```python
from build123d import *

# Parameters (mm, degrees)
SKETCH2_R           = 14.5
BOSS_EXTRUDE1_DEPTH = 14
SKETCH3_W           = 4
SKETCH3_H           = 27
BOSS_EXTRUDE2_DEPTH = 12.3
CUT_EXTRUDE1_DEPTH  = 12.3
SKETCH5_R           = 11
BOSS_EXTRUDE3_DEPTH = 4
SKETCH6_W           = 29
SKETCH6_H           = 36.6
BOSS_EXTRUDE4_DEPTH = 50
FILLET1_R           = 0.2


with BuildPart() as part:
    # Sketch2 → Boss-Extrude1 (new body)
    with BuildSketch(Plane(origin=(0, 0, 0), x_dir=(1, 0, 0), z_dir=(0, 1, 0))):
        with Locations(Location((0, 0, 0), (0, 0, 270))):
            Circle(SKETCH2_R)
    extrude(amount=BOSS_EXTRUDE1_DEPTH)

    # Sketch3 → Boss-Extrude2 (add)
    with BuildSketch(Plane(origin=(0, 14, 0), x_dir=(1, 0, 0), z_dir=(0, 1, 0))):
        Rectangle(SKETCH3_W, SKETCH3_H)
    extrude(amount=BOSS_EXTRUDE2_DEPTH)

    # Sketch4 → Cut-Extrude1 (cut)
    with BuildSketch(Plane(origin=(2, 0, 0), x_dir=(0, 0, -1), z_dir=(1, 0, 0))):
        Polygon((-13.5, 26.3), (-13.5, 14), (-11, 26.3), align=None)
        Polygon((11, 26.3), (13.5, 26.3), (13.5, 14), align=None)
    extrude(amount=-CUT_EXTRUDE1_DEPTH, mode=Mode.SUBTRACT)

    # Sketch5 → Boss-Extrude3 (add)
    with BuildSketch(Plane.XZ):
        with Locations(Location((0, 0, 0), (0, 0, 90))):
            Circle(SKETCH5_R)
    extrude(amount=BOSS_EXTRUDE3_DEPTH)

    # Sketch6 → Boss-Extrude4 (add)
    with BuildSketch(Plane.XZ.offset(4)):
        Rectangle(SKETCH6_W, SKETCH6_H)
    extrude(amount=BOSS_EXTRUDE4_DEPTH)

    # Fillet1
    fillet1_edges = [part.edges().sort_by_distance(p)[0] for p in [
        (2, 26.3, 0),
        (-2, 20.15, 12.25),
        (2, 20.15, 12.25),
        (-2, 26.3, 0),
        (-2, 20.15, -12.25),
        (2, 20.15, -12.25),
        (0, 14, -14.5),
    ]]
    fillet(fillet1_edges, radius=FILLET1_R)


solid = part.part
```
Verification items for the finished model (mm, model axes). A direction names the side the tool comes from. Coordinates: 2 decimals unless noted, no trailing zeros. Order: outer loops, then holes, each group sorted by start corner. A loop starts at its lowest first (then second) coordinate and runs counter-clockwise, first axis right, second up. Notation, with made-up numbers: (-37, -23.75) - (-18, -23.75) arc R22 ccw to (-18, -4.75) - close; hole circle Ø11 at (61, -4.75). An arc over 180 degrees is marked (long way). Return JSON: item names as keys, results as strings.
(1) Go/stop test with flat-tipped pins: pin 1 (3 mm diameter, centred on y = -0.5, z = 10.5, fed in from -X); pin 2 (9.5 mm diameter, centred on y = 19.5, z = 1.5, fed in from -X); pin 3 (9.5 mm diameter, centred on y = 19.5, z = 5.5, fed in from +X). Record where each tip stops, or that it passes through.
Filled sheet:
{"pin 1": "stops at x = -11.3", "pin 2": "stops at x = -2", "pin 3": "stops at x = 2"}
(2) Section check A-A, the plane x = 0. Record the cut outline in (y, z), and give its area (3 significant figures).
Filled sheet:
{"outline": "(-54, -18.3) - (-4, -18.3) - (-4, -11) - (0, -11) - (0, -14.5) - (13.8, -14.5) arc R0.2 ccw to (14, -14.3) - (14, -13.5) - (26.3, -11) - (26.3, 11) - (14, 13.5) - (14, 14.3) arc R0.2 ccw to (13.8, 14.5) - (0, 14.5) - (0, 11) - (-4, 11) - (-4, 18.3) - (-54, 18.3) - close", "area": "2,630 mm^2"}
(3) Access from +Z, -Z, +X, -X, +Y, -Y to the whole of each face (thin tool, end or side, straight path). Record for faces 1 (the flat face through (11, 0, -2)), 2 (the flat face through (0.03, 20.06, 12.27)), 3 (the cylindrical face through (-5.554, 6.803, 13.394)), 4 (the flat face through (0.03, 20.06, -12.27)), 5 (the flat face through (2, 20, 0)).
Filled sheet:
{"face 1": "none", "face 2": "+Z, +X, -X, +Y", "face 3": "+Y", "face 4": "-Z, +X, -X, +Y", "face 5": "+Z, -Z, +X, +Y"}
(4) Section check B-B, the plane z = 0. Record the cut outline in (x, y), and give its area (3 significant figures).
Filled sheet:
{"outline": "(-14.5, -54) - (14.5, -54) - (14.5, -4) - (11, -4) - (11, 0) - (14.5, 0) - (14.5, 13.8) arc R0.2 ccw to (14.3, 14) - (2, 14) - (2, 26.1) arc R0.2 ccw to (1.8, 26.3) - (-1.8, 26.3) arc R0.2 ccw to (-2, 26.1) - (-2, 14) - (-14.3, 14) arc R0.2 ccw to (-14.5, 13.8) - (-14.5, 0) - (-11, 0) - (-11, -4) - (-14.5, -4) - close", "area": "1,990 mm^2"}
(5) Mould release check, pull along Y, two halves, no side actions. Record for faces 6 (the flat face through (0, -4, -12)), 7 (the flat face through (-3, 14, 0)), 8 (the flat face through (-2, 20, 0)): pulls with the +Y half, pulls with the -Y half, needs draft (parallel to the pull), parting line crosses it, or undercut.
Filled sheet:
{"face 6": "undercut", "face 7": "pulls with the +Y half", "face 8": "needs draft"}
(6) Thickness scan on line 1 along Y through (x, z) = (-8.5, 7.5); line 2 along Y through (x, z) = (-6.5, 15); line 3 along Y through (x, z) = (4, 10). Record the ranges inside material, lowest first.
Filled sheet:
{"line 1": "y = -54 to -4, 0 to 14", "line 2": "y = -54 to -4", "line 3": "y = -54 to 14"}
